The listing builds one solid part. Answer for the finished solid, in the listing's coordinates (mm). Face numbers are marked on the shaded views. Give positions to 0.01 mm unless a question says otherwise; leave off trailing zeros. Write each loop counter-clockwise with the first axis right and the second up, starting at its lowest first coordinate (ties: lowest second). Pieces come first, ordered by that corner, then holes.
```python
from build123d import *

# Parameters (mm, degrees)
SKETCH1_W           = 60
SKETCH1_H           = 100
SKETCH1_R           = 7
BOSS_EXTRUDE1_DEPTH = 10
SKETCH2_R           = 6
BOSS_EXTRUDE2_DEPTH = 100


with BuildPart() as part:
    # Sketch1 → Boss-Extrude1 (new body)
    with BuildSketch(Plane.XY):
        Rectangle(SKETCH1_W, SKETCH1_H)
        with Locations((0, -30)):
            Circle(SKETCH1_R, mode=Mode.SUBTRACT)
    extrude(amount=BOSS_EXTRUDE1_DEPTH)

    # Sketch2 → Boss-Extrude2 (add)
    with BuildSketch(Plane.XY.offset(10)):
        with Locations(Location((0, 30, 0), (0, 0, 180))):
            Circle(SKETCH2_R)
    extrude(amount=BOSS_EXTRUDE2_DEPTH)


solid = part.part
```
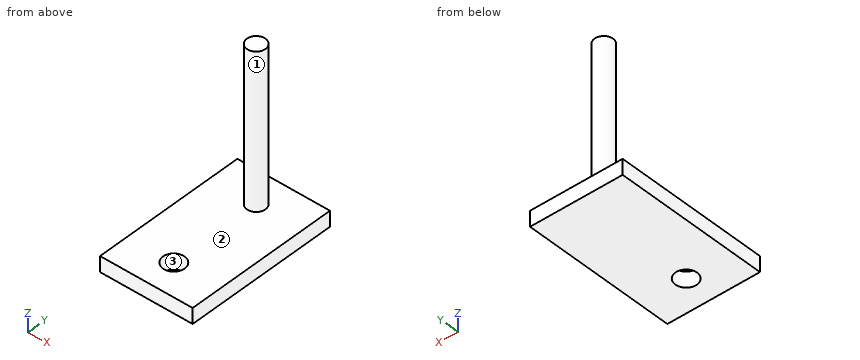
Item 1: Determine the mould class of the marked faces 1, 2 and 3 for opening direction Y: pulls with the +Y half, pulls with the -Y half, needs draft (parallel to the pull), parting line crosses it, or undercut.
Conclusion:
face 1: parting line crosses it
face 2: needs draft
face 3: undercut
Item 2: A cutting plane is placed at B-B, the plane y = -30. Give the vertices of the cut face in (x, z).
Conclusion:
outline: (-30, 0) - (-7, 0) - (-7, 10) - (-30, 10) - close; (7, 0) - (30, 0) - (30, 10) - (7, 10) - close
Item 3: A cutting plane is placed at C-C, the plane y = 27.5. Give the vertices of the cut face in (x, z), plus the area to 3 significant figures.
Conclusion:
outline: (-30, 0) - (30, 0) - (30, 10) - (5.45, 10) - (5.45, 110) - (-5.45, 110) - (-5.45, 10) - (-30, 10) - close
area: 1,690 mm2
Item 4: Consider probe 1 along Y at (x, z) = (0, 7.75); probe 2 along Z at (x, y) = (-22, 33); probe 3 along Y at (x, z) = (-3, 69.5). Determine where each line is inside the solid, lowest interval first.
Conclusion:
probe 1: y = -50 to -37, -23 to 50
probe 2: z = 0 to 10
probe 3: y = 24.8 to 35.2
Item 5: Each of these flat-tipped pins is pushed along its axis until it touches: P1, Ø18, axis at x = 10, y = 23, coming from the +Z side; P2, Ø1.5, axis at y = 26.5, z = 71.5, coming from the +X side; P3, Ø22.5, axis at x = 0, y = -30, coming from the +Z side. Where does it stop, or does it pass through?
Conclusion:
P1: stops at z = 110
P2: stops at x = 5.33
P3: stops at z = 10
Item 6: A cutting plane is placed at D-D, the plane x = 14.5. Give the vertices of the cut face in (y, z), plus the area to 3 significant figures.
Conclusion:
outline: (-50, 0) - (50, 0) - (50, 10) - (-50, 10) - close
area: 1,000 mm2
Item 7: A cutting plane is placed at A-A, the plane x = 2. Give the vertices of the cut face in (y, z), plus the area to 3 significant figures.
Conclusion:
outline: (-50, 0) - (-36.71, 0) - (-36.71, 10) - (-50, 10) - close; (-23.29, 0) - (50, 0) - (50, 10) - (35.66, 10) - (35.66, 110) - (24.34, 110) - (24.34, 10) - (-23.29, 10) - close
area: 2,000 mm2
